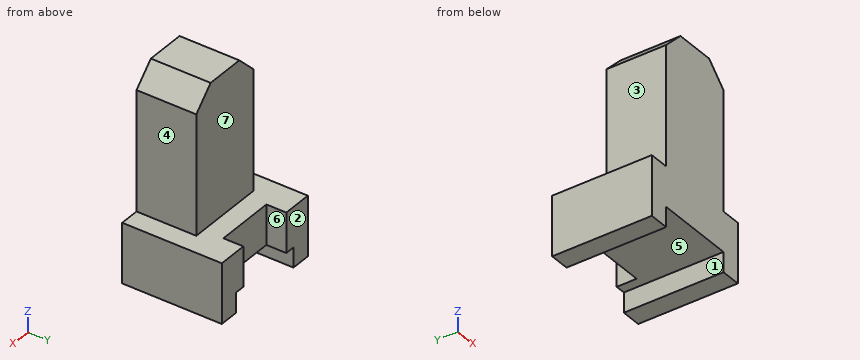
from build123d import *

# Parameters (mm, degrees)
CHAMFERED_BASE_BLOCK_DEPTH = 50
STEP_CUT_SKETCH_W          = 30
STEP_CUT_SKETCH_H          = 40
STEP_CUT_30X40_DEPTH       = 10
UPRIGHT_PROFILE_SKETCH_W   = 40
UPRIGHT_PROFILE_SKETCH_H   = 70
UPRIGHT_BLOCK_DEPTH        = 30
TOP_SLOT_CUT_DEPTH         = 30


with BuildPart() as part:
    # Base Profile Sketch → Chamfered Base Block (new body)
    with BuildSketch(Plane(origin=(0, 0, 0), x_dir=(1, 0, 0), z_dir=(0, 1, 0))):
        Polygon((0, 30), (0, 0), (60, 0), (60, 30), (50, 30), (50, 20), (26.160458453, 20), (10, 20), (10, 30), align=None)
    extrude(amount=CHAMFERED_BASE_BLOCK_DEPTH)

    # Step Cut Sketch → Step Cut 30x40 (cut)
    with BuildSketch(Plane(origin=(0, 50, 0), x_dir=(1, 0, 0), z_dir=(0, 1, 0))):
        with Locations((30, 0)):
            Rectangle(STEP_CUT_SKETCH_W, STEP_CUT_SKETCH_H)
    extrude(amount=-STEP_CUT_30X40_DEPTH, mode=Mode.SUBTRACT)

    # Upright Profile Sketch → Upright Block (add)
    with BuildSketch(Plane.XZ):
        with Locations((30, 35)):
            Rectangle(UPRIGHT_PROFILE_SKETCH_W, UPRIGHT_PROFILE_SKETCH_H)
    extrude(amount=-UPRIGHT_BLOCK_DEPTH)

    # Slot Sketch → Top Slot Cut (cut)
    with BuildSketch(Plane.XZ):
        Polygon((50, 60), (40, 70), (50, 70), align=None)
        Polygon((10, 70), (10, 60), (20, 70), align=None)
    extrude(amount=-TOP_SLOT_CUT_DEPTH, mode=Mode.SUBTRACT)


solid = part.part
Build history of the part. All positions in model axes, mm. Face numbers are marked on the shaded views. A direction names the side the tool comes from. Coordinates: 2 decimals unless noted, no trailing zeros. Order: outer loops, then holes, each group sorted by start corner. A loop starts at its lowest first (then second) coordinate and runs counter-clockwise, first axis right, second up. Notation, with made-up numbers: (-14.75, 82) - (23.25, 82) arc R15 ccw to (23.25, 108) - close; hole circle Ø8 at (29, -1). An arc over 180 degrees is marked (long way). Write item = value, one per line. Start each with the question number.
1) Saw through at C-C on z = 32.5. Write the cut outline in (x, y), then the cut area to 3 significant figures.
2) Wall check: line 1 along X through (y, z) = (8.5, 57); line 2 along Z through (x, y) = (8.5, 2); line 3 along Z through (x, y) = (48, 32). Give the ranges that are in metal, low to high. Write a range as from..to.
3) Two-plate mould, pull along X, no slides. Class the marked faces 1, 2 and 3: pulls with the +X half, pulls with the -X half, needs draft (parallel to the pull), parting line crosses it, or undercut.
4) 3-axis set-ups, long thin cutter, end or side, ignore diameter. For the marked faces 4, 5, 6 and 7: which of +Z, -Z, +X, -X, +Y, -Y reach the whole face in a straight line?
5) Saw through at D-D on y = 34.5. Write the cut outline in (x, z), then the cut area to 3 significant figures.
6) Saw through at A-A on x = 16.5. Write the cut outline in (y, z), then the cut area to 4 significant figures.
7) Saw through at B-B on y = 21.5. Write the cut outline in (x, z).
8) Flat gauge pins, fed straight in: pin 1 Ø22 at (x, z) = (29, -5.5) entering from +Y; pin 2 Ø10 at (x, z) = (19.5, -8.5) entering from -Y; pin 3 Ø3 at (x, y) = (33, 25) entering from -Z; pin 4 Ø24 at (y, z) = (17.5, 16.5) entering from -X. Where does each tip first touch, or does it go through?
From the geometry:
q1.outline = (10, 0) - (50, 0) - (50, 30) - (10, 30) - close
q1.area = 1,200 mm^2
q2.line_1 = 10..50
q2.line_2 = -30..0
q2.line_3 = -20..0
q3.face_1 = undercut
q3.face_2 = needs draft
q3.face_3 = pulls with the -X half
q4.face_4 = +Z, +X, +Y, -Y
q4.face_5 = -Z, +Y, -Y
q4.face_6 = +Z, -Z, +Y
q4.face_7 = +Z, +X, -X, +Y
q5.outline = (0, -30) - (10, -30) - (10, -20) - (50, -20) - (50, -30) - (60, -30) - (60, 0) - (0, 0) - close
q5.area = 1,400 mm^2
q6.outline = (0, -20) - (40, -20) - (40, 0) - (30, 0) - (30, 66.5) - (0, 66.5) - close
q6.area = 2,795 mm^2
q7.outline = (0, -30) - (10, -30) - (10, -20) - (50, -20) - (50, -30) - (60, -30) - (60, 0) - (50, 0) - (50, 60) - (40, 70) - (20, 70) - (10, 60) - (10, 0) - (0, 0) - close
q8.pin_1 = 40
q8.pin_2 = 0
q8.pin_3 = -20
q8.pin_4 = 10
